Geometry: final body of the model. Coordinates: model frame, mm. Coordinates: 2 decimals unless noted, no trailing zeros. Loops run counter-clockwise (first coordinate to the right, second up) from the corner with the lowest first, then second, coordinate; pieces in that order, holes last. Notation, with made-up numbers: (-20, -7.75) - (-15, -7.75) arc R9 ccw to (-15, 8.25) - close; hole circle Ø8 at (43.5, 52.25). An arc over 180 degrees is marked (long way). Answer in a Markdown table with one row per item.
from build123d import *

# Parameters (mm, degrees)
SKETCH1_R             = 25
BOSS_EXTRUDE1_DEPTH   = 112
M8_TAPPED_HOLE1_D     = 6.8
M8_TAPPED_HOLE1_DEPTH = 22
M8_TAPPED_HOLE1_TIP   = 2.042926105
M8_TAPPED_HOLE2_D     = 6.8
M8_TAPPED_HOLE2_DEPTH = 23.75
M8_TAPPED_HOLE2_TIP   = 2.042926105
CHAMFER1_SIZE         = 1


with BuildPart() as part:
    # Sketch1 → Boss-Extrude1 (new body)
    with BuildSketch(Plane.XY):
        Circle(SKETCH1_R)
    extrude(amount=BOSS_EXTRUDE1_DEPTH)

    # M8 Tapped Hole1
    with Locations(Plane.XY.offset(112)):
        with Locations((0, 0)):
            Hole(M8_TAPPED_HOLE1_D / 2, depth=M8_TAPPED_HOLE1_DEPTH)
            with Locations((0, 0, -(M8_TAPPED_HOLE1_DEPTH + M8_TAPPED_HOLE1_TIP / 2))):  # 118° drill point
                Cone(0, M8_TAPPED_HOLE1_D / 2, M8_TAPPED_HOLE1_TIP, mode=Mode.SUBTRACT)

    # M8 Tapped Hole2
    with Locations(Plane(origin=(0, 0, 0), x_dir=(-1, 0, 0), z_dir=(0, 0, -1))):
        with Locations((0, 0)):
            Hole(M8_TAPPED_HOLE2_D / 2, depth=M8_TAPPED_HOLE2_DEPTH)
            with Locations((0, 0, -(M8_TAPPED_HOLE2_DEPTH + M8_TAPPED_HOLE2_TIP / 2))):  # 118° drill point
                Cone(0, M8_TAPPED_HOLE2_D / 2, M8_TAPPED_HOLE2_TIP, mode=Mode.SUBTRACT)

    # Chamfer1
    chamfer1_edges = [part.edges().sort_by_distance(p)[0] for p in [
        (-25, 0, 0),
        (-25, 0, 112),
    ]]
    chamfer(chamfer1_edges, length=CHAMFER1_SIZE)


solid = part.part
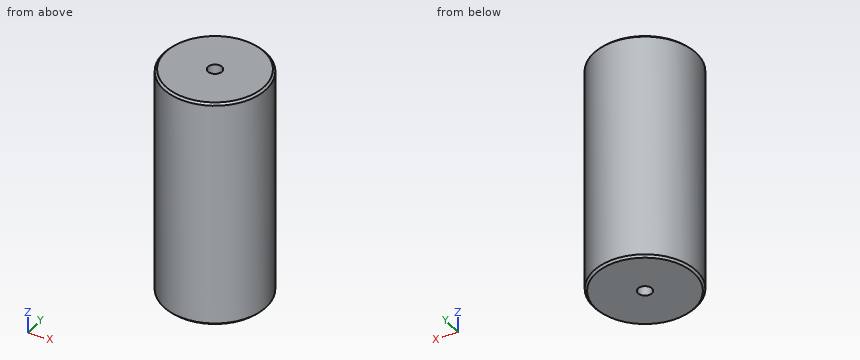
(1) First-contact query: pin 1 Ø10 at (y, z) = (16.5, 60.5) entering from +X; pin 2 Ø1 at (x, z) = (-12, 94.5) entering from +Y; pin 3 Ø5 at (x, z) = (8, 75.5) entering from -Y. Flat tips, straight axial feed; report the tip coordinate or a pass-through.
Verdict:
| item | result |
|---|---|
| pin 1 | stops at x = 22.2 |
| pin 2 | stops at y = 22.2 |
| pin 3 | stops at y = -24.39 |
(2) Ray query, probe 1 along Y at (x, z) = (0, 8); probe 2 along X at (y, z) = (-7, 13); probe 3 along Y at (x, z) = (-16.5, 97). Return the intervals inside material, ascending.
Verdict:
| item | result |
|---|---|
| probe 1 | y = -25 to -3.4, 3.4 to 25 |
| probe 2 | x = -24 to 24 |
| probe 3 | y = -18.78 to 18.78 |
(3) Cut plane B-B on z = 103. Output: boundary loops of the cut face in (x, y), then the cut area to 3 significant figures.
Verdict:
| item | result |
|---|---|
| outline | circle Ø50 at (0, 0); hole circle Ø6.8 at (0, 0) |
| area | 1,930 mm² |
(4) Cut plane A-A on z = 29.5. Output: boundary loops of the cut face in (x, y).
Verdict:
| item | result |
|---|---|
| outline | circle Ø50 at (0, 0) |
